Model file for the job. Use its own axes, mm. A direction names the side the tool comes from. Round coordinates to 2 decimals unless told otherwise and drop trailing zeros. Loops run counter-clockwise (first coordinate to the right, second up) from the corner with the lowest first, then second, coordinate; pieces in that order, holes last. Notation, with made-up numbers: M -12.75,-8 L -6.75,-8 A25 ccw -6.75,20 Z; hole C 49,28 d11. An arc over 180 degrees is marked long. Use a Markdown table: item, result. Add a question column.
Q1. Pin check, flat tips, straight feed: pin 1 (1.5 mm diameter, centred on x = 507.5, z = -1557.5, fed in from +Y); pin 2 (1 mm diameter, centred on y = 203, z = -1557, fed in from +X); pin 3 (2 mm diameter, centred on x = 527, z = -1565, fed in from -Y). Stop position of each tip, or through.
Q2. Probe line 1 (Y direction, x = 522, z = -1565.5); line 2 (X direction, y = 230, z = -1568.25); line 3 (X direction, y = 245, z = -1565.25). List the from-to ranges inside material, lowest first. Write a range as from..to.
Q3. Tool access for faces 1 (the face through (483.95, 240.34, -1559.86)), 2 (the face through (537.825, 268.668, -1559.858)), 3 (the face through (555.15, 218.15, -1559.86)), 4 (the face through (504.637, 200.82, -1559.858)), 5 (the face through (487.307, 251.338, -1559.858)): list every direction of +Z, -Z, +X, -X, +Y, -Y with a clear straight run to the whole face (end or side of a thin tool).
Q4. Mould opens along X. For faces 6 (the face through (556.814, 253.014, -1559.858)), 7 (the face through (485.65, 216.47, -1559.86)), 8 (the face through (499.77, 227.99, -1559.86)) say: +X half, -X half, draft (parallel to the pull), parting line (faces both ways), or undercut.
Q5. Cut at A-A (y = 236). Give the cut face in (x, z).
Q6. Cut at B-B (x = 533.5). Give the cut face in (y, z).
Q7. Cut at D-D (x = 493.5). Give the cut face in (y, z).
Q8. Cut at C-C (z = -1555.5). Give the cut face in (x, y).
from build123d import *

# Parameters (mm, degrees)
SKETCH1_R           = 22.5
BOSS_EXTRUDE1_DEPTH = 20


with BuildPart() as part:
    # Sketch1 → Boss-Extrude1 (new body)
    with BuildSketch(Plane.XY.offset(-1549.998443067)):
        with BuildLine():
            Line((526.153967379, 269.86978568), (527.517933611, 274.246748006))
            ThreePointArc((527.517933611, 274.246748006), (502.642081617, 270.162396725), (485.149256781, 252.010509299))
            Line((485.149256781, 252.010509299), (489.526219107, 250.646543068))
            Line((489.526219107, 250.646543068), (486.104820559, 239.667288449))
            Line((486.104820559, 239.667288449), (481.727858233, 241.031254681))
            ThreePointArc((481.727858233, 241.031254681), (485.812209514, 216.155402687), (503.964096939, 198.662577851))
            Line((503.964096939, 198.662577851), (505.328063171, 203.039540177))
            Line((505.328063171, 203.039540177), (516.307317789, 199.618141629))
            Line((516.307317789, 199.618141629), (514.943351558, 195.241179303))
            ThreePointArc((514.943351558, 195.241179303), (539.819203552, 199.325530584), (557.312028388, 217.47741801))
            Line((557.312028388, 217.47741801), (552.935066061, 218.841384241))
            Line((552.935066061, 218.841384241), (556.35646461, 229.82063886))
            Line((556.35646461, 229.82063886), (560.733426936, 228.456672628))
            ThreePointArc((560.733426936, 228.456672628), (556.649075655, 253.332524622), (538.497188229, 270.825349458))
            Line((538.497188229, 270.825349458), (537.133221997, 266.448387132))
            Line((537.133221997, 266.448387132), (526.153967379, 269.86978568))
        make_face()
        with Locations(Location((521.230642584, 234.743963655, 0), (0, 0, 180))):
            Circle(SKETCH1_R, mode=Mode.SUBTRACT)
    extrude(amount=-BOSS_EXTRUDE1_DEPTH)


solid = part.part
Checked values:
| question | item | result |
|---|---|---|
| 1 | pin 1 | stops at y = 272.58 |
| 1 | pin 2 | stops at x = 546.21 |
| 1 | pin 3 | stops at y = 195.03 |
| 2 | line 1 | y = 194.75..212.26, 257.23..274.74 |
| 2 | line 2 | x = 481.51..499.24, 543.22..560.95 |
| 2 | line 3 | x = 487.77..501.2, 541.26..559.89 |
| 3 | face 1 | +Z, -Z |
| 3 | face 2 | +Z, -Z, +Y |
| 3 | face 3 | +Z, -Z, +X |
| 3 | face 4 | +Z, -Z, -Y |
| 3 | face 5 | +Z, -Z, -X |
| 4 | face 6 | +X half |
| 4 | face 7 | -X half |
| 4 | face 8 | undercut |
| 5 | outline | M 481.25,-1570 L 498.77,-1570 L 498.77,-1550 L 481.25,-1550 Z; M 543.7,-1570 L 561.21,-1570 L 561.21,-1550 L 543.7,-1550 Z |
| 6 | outline | M 196.67,-1570 L 215.88,-1570 L 215.88,-1550 L 196.67,-1550 Z; M 253.6,-1570 L 267.58,-1570 L 267.58,-1550 L 253.6,-1550 Z |
| 7 | outline | M 205.92,-1570 L 263.57,-1570 L 263.57,-1550 L 205.92,-1550 Z |
| 8 | outline | M 481.73,241.03 A40 ccw 503.96,198.66 L 505.33,203.04 L 516.31,199.62 L 514.94,195.24 A40 ccw 557.31,217.48 L 552.94,218.84 L 556.36,229.82 L 560.73,228.46 A40 ccw 538.5,270.83 L 537.13,266.45 L 526.15,269.87 L 527.52,274.25 A40 ccw 485.15,252.01 L 489.53,250.65 L 486.1,239.67 Z; hole C 521.23,234.74 d45 |
